from build123d import *

# Parameters (mm, degrees)
SKETCH1_W                  = 250
SKETCH1_H                  = 175
BOSS_EXTRUDE1_DEPTH        = 25
CUT_EXTRUDE1_DEPTH         = 155.616460961
SKETCH3_R                  = 16
CUT_EXTRUDE2_DEPTH         = 155.616460961
M5_TAPPED_HOLE2_AT_2_COUNT = 2
M5_TAPPED_HOLE2_AT_2_PITCH = 24
M5_TAPPED_HOLE2_AT_3_COUNT = 2
M5_TAPPED_HOLE2_AT_3_PITCH = 36
M5_TAPPED_HOLE2_AT_4_COUNT = 2
M5_TAPPED_HOLE2_AT_4_PITCH = 43.266615306
SKETCH7_R                  = 25
CUT_EXTRUDE3_DEPTH         = 155.616460961
M5_TAPPED_HOLE1_D          = 4.2


with BuildPart() as part:
    # Sketch1 → Boss-Extrude1 (new body)
    with BuildSketch(Plane(origin=(0, 0, 0), x_dir=(1, 0, 0), z_dir=(0, 1, 0))):
        Rectangle(SKETCH1_W, SKETCH1_H)
    extrude(amount=BOSS_EXTRUDE1_DEPTH)

    # Sketch2 → Cut-Extrude1 (cut, through all)
    with BuildSketch(Plane(origin=(0, 25, 0), x_dir=(1, 0, 0), z_dir=(0, 1, 0))):
        with BuildLine():
            Line((-20, -47.5), (-20, -87.5))
            Line((-20, -87.5), (20, -87.5))
            Line((20, -87.5), (20, -47.5))
            ThreePointArc((20, -47.5), (0, -27.5), (-20, -47.5))
        make_face()
    extrude(amount=-CUT_EXTRUDE1_DEPTH, mode=Mode.SUBTRACT)

    # Sketch3 → Cut-Extrude2 (cut, through all)
    with BuildSketch(Plane(origin=(0, 25, 0), x_dir=(1, 0, 0), z_dir=(0, 1, 0))):
        with Locations(Location((-80, 57.5, 0), (0, 0, 270))):
            Circle(SKETCH3_R)
        with Locations(Location((80, 57.5, 0), (0, 0, 90))):
            Circle(SKETCH3_R)
    extrude(amount=-CUT_EXTRUDE2_DEPTH, mode=Mode.SUBTRACT)

    # Sketch6 → M5 Tapped Hole2 (revolve, cut)
    with BuildSketch(Plane(origin=(-92, 25, -75.5), x_dir=(0, 0, 1), z_dir=(1, 0, 0))):
        Polygon((0, 0), (0, 13.6618073), (2.1, 12.4), (2.1, 0), align=None)
    m5_tapped_hole2 = revolve(axis=Axis((-92, 31.35, -75.5), (0, -1, 0)), mode=Mode.SUBTRACT)

    # M5 Tapped Hole2 at 2: M5 Tapped Hole2 ×2
    with Locations(*[(i * M5_TAPPED_HOLE2_AT_2_PITCH, 0, 0) for i in range(1, M5_TAPPED_HOLE2_AT_2_COUNT)]):
        add(m5_tapped_hole2, mode=Mode.SUBTRACT)

    # M5 Tapped Hole2 at 3: M5 Tapped Hole2 ×2
    with Locations(*[(0, 0, i * M5_TAPPED_HOLE2_AT_3_PITCH) for i in range(1, M5_TAPPED_HOLE2_AT_3_COUNT)]):
        add(m5_tapped_hole2, mode=Mode.SUBTRACT)

    # M5 Tapped Hole2 at 4: M5 Tapped Hole2 ×2
    with Locations(*[Vector(0.5547001962252294, 0, 0.8320502943378435) * (i * M5_TAPPED_HOLE2_AT_4_PITCH) for i in range(1, M5_TAPPED_HOLE2_AT_4_COUNT)]):
        add(m5_tapped_hole2, mode=Mode.SUBTRACT)

    # Mirror1: M5 Tapped Hole2 across plane
    add(m5_tapped_hole2.mirror(Plane(origin=(0, 0, 0), x_dir=(0, 0, 1), z_dir=(1, 0, 0))), mode=Mode.SUBTRACT)

    # Mirror1 copy 1 sketch → Mirror1 copy 1 (revolve, cut)
    with BuildSketch(Plane(origin=(68, 25, -75.5), x_dir=(0, 0, 1), z_dir=(-1, 0, 0))):
        Polygon((0, 0), (0, -13.6618073), (2.1, -12.4), (2.1, 0), align=None)
    revolve(axis=Axis((68, 31.35, -75.5), (0, 1, 0)), mode=Mode.SUBTRACT)

    # Mirror1 copy 2 sketch → Mirror1 copy 2 (revolve, cut)
    with BuildSketch(Plane(origin=(92, 25, -39.5), x_dir=(0, 0, 1), z_dir=(-1, 0, 0))):
        Polygon((0, 0), (0, -13.6618073), (2.1, -12.4), (2.1, 0), align=None)
    revolve(axis=Axis((92, 31.35, -39.5), (0, 1, 0)), mode=Mode.SUBTRACT)

    # Mirror1 copy 3 sketch → Mirror1 copy 3 (revolve, cut)
    with BuildSketch(Plane(origin=(68, 25, -39.5), x_dir=(0, 0, 1), z_dir=(-1, 0, 0))):
        Polygon((0, 0), (0, -13.6618073), (2.1, -12.4), (2.1, 0), align=None)
    revolve(axis=Axis((68, 31.35, -39.5), (0, 1, 0)), mode=Mode.SUBTRACT)

    # Sketch7 → Cut-Extrude3 (cut, through all)
    with BuildSketch(Plane(origin=(0, 25, 0), x_dir=(1, 0, 0), z_dir=(0, 1, 0))):
        with Locations(Location((0, 57.5, 0), (0, 0, 270))):
            Circle(SKETCH7_R)
    extrude(amount=-CUT_EXTRUDE3_DEPTH, mode=Mode.SUBTRACT)

    # M5 Tapped Hole1 (through all)
    with Locations(Plane(origin=(0, 25, 0), x_dir=(1, 0, 0), z_dir=(0, 1, 0))):
        with Locations((-31, 57.5), (31, 57.5)):
            Hole(M5_TAPPED_HOLE1_D / 2)


solid = part.part
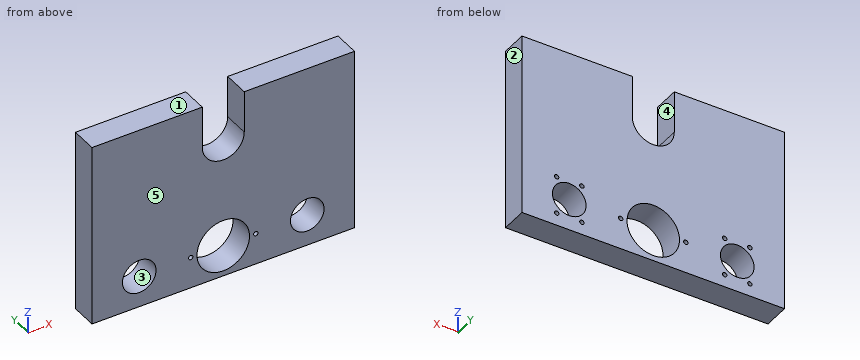
Design review of the part built by this model. Coordinates are the model's own, in mm. Face numbers are marked on the shaded views. A direction names the side the tool comes from. Coordinates: 2 decimals unless noted, no trailing zeros. Order: outer loops, then holes, each group sorted by start corner. A loop starts at its lowest first (then second) coordinate and runs counter-clockwise, first axis right, second up.
Item 1: For line 1 (X direction, y = 11, z = -57.5); line 2 (Z direction, x = 80, y = 20.75); line 3 (X direction, y = 21, z = -39.5), list the stretches that pass through material, from the lowest coordinate up.
Item 2: For pin 1 Ø3.5 at (x, z) = (-68, -75.5) entering from +Y; pin 2 Ø4 at (x, z) = (92, -39.5) entering from +Y, all flat-tipped, find the tip position at first contact; note any pin that passes through.
Item 3: For the marked faces 4 and 5, list the 3-axis set-ups (+Z, -Z, +X, -X, +Y, -Y) from which the entire face can be reached by the end or side of a thin tool; tool diameter is ignored.
Item 4: Take a section at A-A, the plane x = 0. Write out the cut boundary in (y, z).
Item 5: Take a section at B-B, the plane z = 75.5. Write out the cut boundary in (x, y).
Item 6: The part is to be moulded in two halves that separate along Z. For the marked faces 1, 2 and 3, say which applies: pulls with the +Z half, pulls with the -Z half, needs draft (parallel to the pull), parting line crosses it, or undercut.
Item 7: Take a section at C-C, the plane y = 20.75. Count the separate pieces of the cut face and the enclosed holes in it, then the cut area to 3 significant figures.
Item 8: Take a section at D-D, the plane y = 8. Write out the cut boundary in (x, z).
The answers:
1. line 1: x = -125 to -96, -64 to -33.1, -28.9 to -25, 25 to 28.9, 33.1 to 64, 96 to 125
1. line 2: z = -87.5 to -73.5, -41.5 to 87.5
1. line 3: x = -125 to -94.1, -89.9 to -70.1, -65.9 to -17.35, 17.35 to 65.9, 70.1 to 89.9, 94.1 to 125
2. pin 1: stops at y = 12.39
2. pin 2: stops at y = 12.54
3. face 4: +Z, +Y, -Y
3. face 5: +Z, -Z, +X, -X, -Y
4. outline: (0, -87.5) - (25, -87.5) - (25, -82.5) - (0, -82.5) - close; (0, -32.5) - (25, -32.5) - (25, 27.5) - (0, 27.5) - close
5. outline: (-125, 0) - (-20, 0) - (-20, 25) - (-125, 25) - close; (20, 0) - (125, 0) - (125, 25) - (20, 25) - close
6. face 1: pulls with the +Z half
6. face 2: needs draft
6. face 3: undercut
7. separate pieces: 1
7. enclosed holes: 13
7. area: 37,800 mm2
8. outline: (-125, -87.5) - (125, -87.5) - (125, 87.5) - (20, 87.5) - (20, 47.5) arc R20 cw to (-20, 47.5) - (-20, 87.5) - (-125, 87.5) - close; hole circle Ø32 at (-80, -57.5); hole circle Ø4.2 at (-31, -57.5); hole circle Ø50 at (0, -57.5); hole circle Ø4.2 at (31, -57.5); hole circle Ø32 at (80, -57.5)
